Design review of the part built by this model. Coordinates are the model's own, in mm. A direction names the side the tool comes from. Coordinates: 2 decimals unless noted, no trailing zeros. Loops run counter-clockwise (first coordinate to the right, second up) from the corner with the lowest first, then second, coordinate; pieces in that order, holes last. Notation, with made-up numbers: (2.5, -6.75) -> (50.5, -6.75) arc R23 ccw to (50.5, 14.25) -> close; hole circle Ø8 at (17.5, 67.5). An arc over 180 degrees is marked (long way). Use a Markdown table: item, result. Add a question column.
Q1. Take a section at A-A on z = 15. Write out the cut boundary in (x, y), plus the area to 3 significant figures.
Q2. For probe 1 along Z at (x, y) = (28, -6.5); probe 2 along Y at (x, z) = (26, 3); probe 3 along X at (y, z) = (-11.75, 21.5), list the stretches that pass through material, from the lowest coordinate up.
Q3. Draft analysis for pull direction Z (two halves, no side actions). For faces 5 (the face through (0.5, -13.9, 25)), 6 (the face through (35, -3, 0)), 7 (the face through (24.767, -3.451, 13.659)), state which applies: pulls with the +Z half, pulls with the -Z half, needs draft (parallel to the pull), parting line crosses it, or undercut.
Q4. Clearance check with flat-ended pins moving along their axes: pin 1 Ø9 at (x, z) = (-28, -15) entering from -Y; pin 2 Ø6 at (x, y) = (0.5, -7.5) entering from +Z; pin 3 Ø4 at (x, z) = (6.5, -2) entering from -Y; pin 4 Ø1.5 at (x, z) = (-1.5, -16) entering from +Y. State where each tip first meets the part, or that it passes through.
Q5. Take a section at B-B on x = -28. Write out the cut boundary in (y, z), plus the area to 3 significant figures.
Q6. Take a section at C-C on y = -11. Write out the cut boundary in (x, z), plus the area to 3 significant figures.
Q7. For faces 1 (the face through (29, -7, 0)), 2 (the face through (-28, -7, 0)), 3 (the face through (6.97, -7.17, 0.35)), 4 (the face through (24, 0, 0)), list the 3-axis set-ups (+Z, -Z, +X, -X, +Y, -Y) from which the entire face can be reached by the end or side of a thin tool; tool diameter is ignored.
Q8. Take a section at D-D on z = -3.5. Write out the cut boundary in (x, y), plus the area to 3 significant figures.
from build123d import *

# Parameters (mm, degrees)
SADDLE_BODY_DEPTH           = 25
FLANGE_MOUNTING_HOLES_REACH = 50.775
FLANGE_HOLES_SKETCH_R       = 3.5


with BuildPart() as part:
    # Saddle Profile Sketch → Saddle Body (new, symmetric)
    with BuildSketch(Plane.XY):
        with BuildLine():
            Line((0, -14.142135624), (14.142135624, 0))
            Line((14.142135624, 0), (35, 0))
            Line((35, 0), (35, -7))
            Line((35, -7), (21.9089023, -7))
            ThreePointArc((21.9089023, -7), (0, -23), (-21.9089023, -7))
            Line((-21.9089023, -7), (-35, -7))
            Line((-35, -7), (-35, 0))
            Line((-35, 0), (-14.142135624, 0))
            Line((-14.142135624, 0), (0, -14.142135624))
        make_face()
    extrude(amount=SADDLE_BODY_DEPTH, both=True)

    # Flange Holes Sketch → Flange Mounting Holes (cut, up to next)
    with BuildSketch(Plane(origin=(0, 0, 0), x_dir=(1, 0, 0), z_dir=(0, 1, 0)), mode=Mode.PRIVATE) as flange_mounting_holes_sk1:
        with Locations(Location((-28, 15, 0), (0, 0, 180))):
            Circle(FLANGE_HOLES_SKETCH_R)
    flange_mounting_holes_tool1 = extrude(flange_mounting_holes_sk1.sketch, amount=-FLANGE_MOUNTING_HOLES_REACH, mode=Mode.PRIVATE) & part.part
    # Flange Holes Sketch → Flange Mounting Holes (cut, up to next)
    with BuildSketch(Plane(origin=(0, 0, 0), x_dir=(1, 0, 0), z_dir=(0, 1, 0)), mode=Mode.PRIVATE) as flange_mounting_holes_sk2:
        with Locations(Location((-28, -15, 0), (0, 0, 180))):
            Circle(FLANGE_HOLES_SKETCH_R)
    flange_mounting_holes_tool2 = extrude(flange_mounting_holes_sk2.sketch, amount=-FLANGE_MOUNTING_HOLES_REACH, mode=Mode.PRIVATE) & part.part
    # Flange Holes Sketch → Flange Mounting Holes (cut, up to next)
    with BuildSketch(Plane(origin=(0, 0, 0), x_dir=(1, 0, 0), z_dir=(0, 1, 0)), mode=Mode.PRIVATE) as flange_mounting_holes_sk3:
        with Locations(Location((28, -15, 0), (0, 0, 180))):
            Circle(FLANGE_HOLES_SKETCH_R)
    flange_mounting_holes_tool3 = extrude(flange_mounting_holes_sk3.sketch, amount=-FLANGE_MOUNTING_HOLES_REACH, mode=Mode.PRIVATE) & part.part
    # Flange Holes Sketch → Flange Mounting Holes (cut, up to next)
    with BuildSketch(Plane(origin=(0, 0, 0), x_dir=(1, 0, 0), z_dir=(0, 1, 0)), mode=Mode.PRIVATE) as flange_mounting_holes_sk4:
        with Locations(Location((28, 15, 0), (0, 0, 180))):
            Circle(FLANGE_HOLES_SKETCH_R)
    flange_mounting_holes_tool4 = extrude(flange_mounting_holes_sk4.sketch, amount=-FLANGE_MOUNTING_HOLES_REACH, mode=Mode.PRIVATE) & part.part
    add(flange_mounting_holes_tool1.solids().sort_by_distance((-28, 0, -15))[0], mode=Mode.SUBTRACT)
    add(flange_mounting_holes_tool2.solids().sort_by_distance((-28, 0, 15))[0], mode=Mode.SUBTRACT)
    add(flange_mounting_holes_tool3.solids().sort_by_distance((28, 0, 15))[0], mode=Mode.SUBTRACT)
    add(flange_mounting_holes_tool4.solids().sort_by_distance((28, 0, -15))[0], mode=Mode.SUBTRACT)


solid = part.part
Answer list:
| question | item | result |
|---|---|---|
| 1 | outline | (-35, -7) -> (-31.5, -7) -> (-31.5, 0) -> (-35, 0) -> close; (-24.5, -7) -> (-21.91, -7) arc R23 ccw to (21.91, -7) -> (24.5, -7) -> (24.5, 0) -> (14.14, 0) -> (0, -14.14) -> (-14.14, 0) -> (-24.5, 0) -> close; (31.5, -7) -> (35, -7) -> (35, 0) -> (31.5, 0) -> close |
| 1 | area | 706 mm² |
| 2 | probe 1 | -25 to -18.5, -11.5 to 11.5, 18.5 to 25 |
| 2 | probe 2 | -7 to 0 |
| 2 | probe 3 | -19.77 to -2.39, 2.39 to 19.77 |
| 3 | face 5 | pulls with the +Z half |
| 3 | face 6 | needs draft |
| 3 | face 7 | undercut |
| 4 | pin 1 | y = -7 |
| 4 | pin 2 | through |
| 4 | pin 3 | y = -22.56 |
| 4 | pin 4 | y = -11.89 |
| 5 | outline | (-7, -25) -> (0, -25) -> (0, -18.5) -> (-7, -18.5) -> close; (-7, -11.5) -> (0, -11.5) -> (0, 11.5) -> (-7, 11.5) -> close; (-7, 18.5) -> (0, 18.5) -> (0, 25) -> (-7, 25) -> close |
| 5 | area | 252 mm² |
| 6 | outline | (-20.2, -25) -> (-3.14, -25) -> (-3.14, 25) -> (-20.2, 25) -> close; (3.14, -25) -> (20.2, -25) -> (20.2, 25) -> (3.14, 25) -> close |
| 6 | area | 1,710 mm² |
| 7 | face 1 | +Z, -Z, +X, -Y |
| 7 | face 2 | +Z, -Z, -X, -Y |
| 7 | face 3 | +Z, -Z, +Y |
| 7 | face 4 | +Z, -Z, +X, -X, +Y |
| 8 | outline | (-35, -7) -> (-21.91, -7) arc R23 ccw to (21.91, -7) -> (35, -7) -> (35, 0) -> (14.14, 0) -> (0, -14.14) -> (-14.14, 0) -> (-35, 0) -> close |
| 8 | area | 804 mm² |
